Study the drawing (mm; zero at the part's minimum x, y, z) and answer. Round coordinates to 2 decimals unless told otherwise and drop trailing zeros. Order: outer loops, then holes, each group sorted by start corner. A loop starts at its lowest first (then second) coordinate and runs counter-clockwise, first axis right, second up. Notation, with made-up numbers: (-39.75, 45.5) - (-19.75, 45.5) arc R19 ccw to (-19.75, 78.5) - close; hole circle Ø11 at (-20.5, 5). An arc over 180 degrees is marked (long way). Put each result on its own line as item: value. Start each with the question number.
Q1. Find the intervals of material crossed by line 1 along X through (y, z) = (7, 26); line 2 along Y through (x, z) = (6.25, 7); line 3 along X through (y, z) = (2.75, 85), in increasing order. Write a range as from..to.
Q2. Each of these flat-tipped pins is pushed along its axis until it touches: pin 1 Ø2 at (x, z) = (8, 33.5) entering from +Y; pin 2 Ø4 at (x, z) = (1.5, 13) entering from -Y; pin 3 Ø4 at (x, z) = (6.5, 68.5) entering from -Y. Where does it stop, or does it pass through?
Q3. Section B-B on z = 86 is taken. Give the vertices of the cut face in (x, y), then the cut area to 3 significant figures.
Q4. Section A-A on x = 7 is taken. Give the vertices of the cut face in (y, z), then the cut area to 3 significant figures.
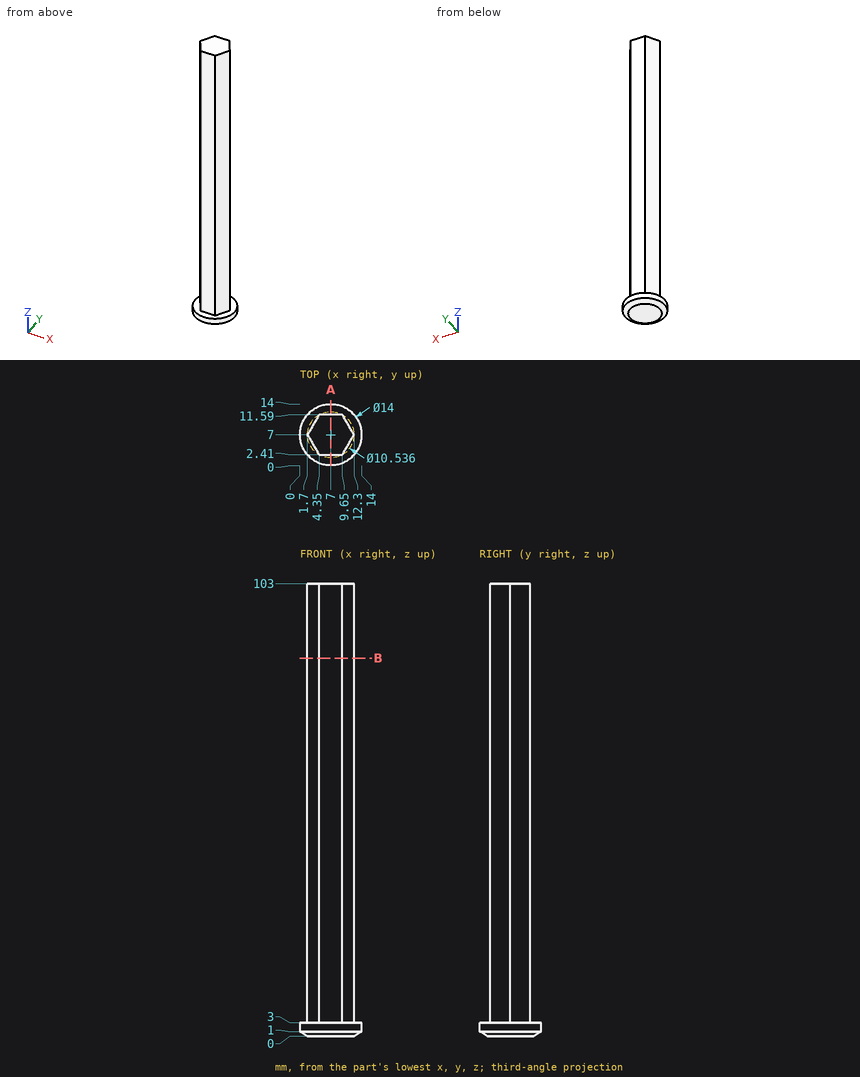
Findings:
1. line 1: 1.7..12.3
1. line 2: 2.41..11.59
1. line 3: 4.15..9.85
2. pin 1: y = 11.59
2. pin 2: y = 3.88
2. pin 3: y = 2.41
3. outline: (1.7, 7) - (4.35, 2.41) - (9.65, 2.41) - (12.3, 7) - (9.65, 11.59) - (4.35, 11.59) - close
3. area: 73.0 mm2
4. outline: (0, 1) - (1.73, 0) - (12.27, 0) - (14, 1) - (14, 3) - (11.59, 3) - (11.59, 103) - (2.41, 103) - (2.41, 3) - (0, 3) - close
4. area: 958 mm2
